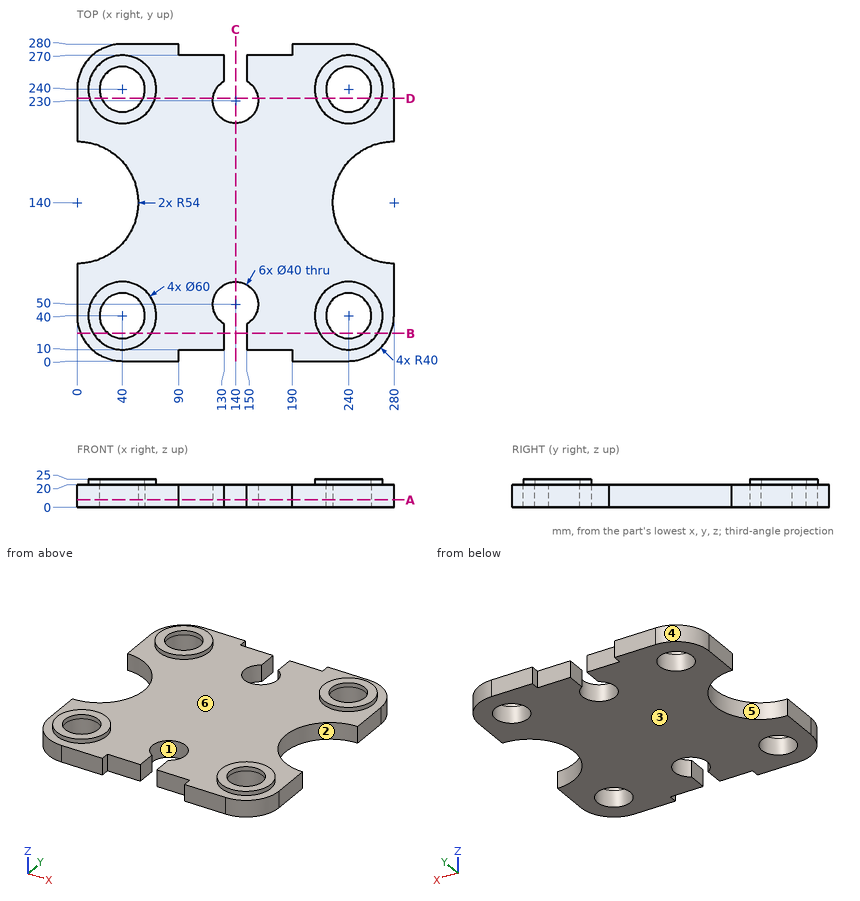
Design review of the part shown in the three views and the two pictorial views. Dimensions are in mm from the part's minimum x, y and z. A direction names the side the tool comes from. Round coordinates to 2 decimals unless told otherwise and drop trailing zeros. Loops run counter-clockwise (first coordinate to the right, second up) from the corner with the lowest first, then second, coordinate; pieces in that order, holes last. Notation, with made-up numbers: M -1,75 L 32,75 A12 ccw 32,96 Z; hole C -1,36.5 d6. An arc over 180 degrees is marked long. Write item = value, one per line.
Item 1: Insertion check: P1, Ø6, axis at x = 101.5, z = 11.5, coming from the +Y side; P2, Ø6, axis at y = 161, z = 6.5, coming from the +X side; P3, Ø4, axis at y = 166, z = 21, coming from the +X side (3 decimals). Each pin has a flat end and moves straight along its axis. Give the tip position at first contact, or say it passes through.
Return value:
P1 = 270
P2 = 231.63
P3 = 233.665
Item 2: Take a section at A-A on z = 6.5. State how many separate pieces and enclosed holes the cut face has, then the cut area to 3 significant figures.
Return value:
separate_pieces = 1
enclosed_holes = 4
area = 57,500 mm2
Item 3: Take a section at D-D on y = 232. Write out the cut boundary in (x, z), then the cut area to 3 significant figures.
Return value:
outline = M 0,0 L 21.67,0 L 21.67,25 L 11.09,25 L 11.09,20 L 0,20 Z; M 58.33,0 L 120.1,0 L 120.1,20 L 68.91,20 L 68.91,25 L 58.33,25 Z; M 159.9,0 L 221.67,0 L 221.67,25 L 211.09,25 L 211.09,20 L 159.9,20 Z; M 258.33,0 L 280,0 L 280,20 L 268.91,20 L 268.91,25 L 258.33,25 Z
area = 3,550 mm2
Item 4: For line 1 (Y direction, x = 240, z = 22.15); line 2 (Y direction, x = 25, z = 9.75); line 3 (X direction, y = 250, z = 4.75), list the stretches that pass through material, from the lowest coordinate up. Write a range as [from, to].
Return value:
line_1 = [10, 20], [60, 70], [210, 220], [260, 270]
line_2 = [2.92, 26.77], [53.23, 92.14], [187.86, 226.77], [253.23, 277.08]
line_3 = [1.27, 22.68], [57.32, 130], [150, 222.68], [257.32, 278.73]
Item 5: Take a section at B-B on y = 24.5. Write out the cut boundary in (x, z).
Return value:
outline = M 3.13,0 L 27.36,0 L 27.36,25 L 14.31,25 L 14.31,20 L 3.13,20 Z; M 52.64,0 L 130,0 L 130,20 L 65.69,20 L 65.69,25 L 52.64,25 Z; M 150,0 L 227.36,0 L 227.36,25 L 214.31,25 L 214.31,20 L 150,20 Z; M 252.64,0 L 276.87,0 L 276.87,20 L 265.69,20 L 265.69,25 L 252.64,25 Z
Item 6: Take a section at C-C on x = 140. Write out the cut boundary in (y, z).
Return value:
outline = M 70,0 L 210,0 L 210,20 L 70,20 Z
Item 7: The part is to be moulded in two halves that separate along X. For the marked faces 1, 2, 3 and 4, say which applies: released by +X, released by -X, zero draft, split by the parting line, or undercut.
Return value:
face_1 = undercut
face_2 = released by +X
face_3 = zero draft
face_4 = released by -X
Item 8: Machinability: for the marked faces 5 and 6, which of the approach directions +Z, -Z, +X, -X, +Y, -Y give a long, thin tool a straight path to every point of the face, cutting with its end or side? Answer none if there is none.
Return value:
face_5 = +Z, -Z, -X
face_6 = +Z
